For this review, take the finished solid that the model builds, in its own axes (mm). Face numbers are marked on the shaded views. A direction names the side the tool comes from. Give positions to 0.01 mm unless a question says otherwise; leave off trailing zeros. Write each loop counter-clockwise with the first axis right and the second up, starting at its lowest first coordinate (ties: lowest second). Pieces come first, ordered by that corner, then holes. Notation, with made-up numbers: M 61.25,69.25 L 94.25,69.25 A30 ccw 94.25,101.25 Z; hole C 25,-11 d10. An arc over 180 degrees is marked long. Write item = value, one per line.
```python
from build123d import *

# Parameters (mm, degrees)
CHAMFER1_SIZE = 0.5


with BuildPart() as part:
    # Sketch1 → Revolve1 (revolve)
    with BuildSketch(Plane.XY, mode=Mode.PRIVATE) as revolve1_sk:
        Polygon((-99.067365632, -10.161784701), (-100.317365632, -10.161784701), (-100.317365632, -13.161784701), (-92.817365632, -13.161784701), (-92.817365632, 8.038215299), (-97.067365632, 8.038215299), (-97.067365632, 0.538215299), (-99.067365632, 0.538215299), align=None)
    revolve(revolve1_sk.sketch.rotate(Axis((-92.817365632, 8.102615299, 0), (0, -1, 0)), 270), axis=Axis((-92.817365632, 8.102615299, 0), (0, -1, 0)))

    # Chamfer1
    chamfer1_edges = [part.edges().sort_by_distance(p)[0] for p in [
        (-92.817365632, 0.538215299, -6.25),
        (-92.817365632, 8.038215299, -4.25),
    ]]
    chamfer(chamfer1_edges, length=CHAMFER1_SIZE)


solid = part.part
```
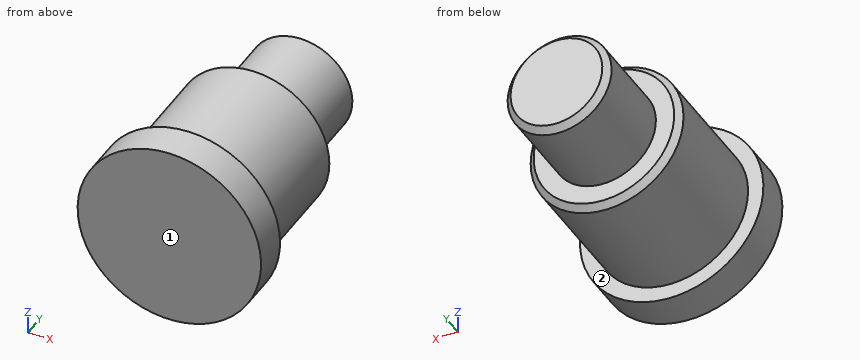
1. We need section A-A, the plane z = 0. Write out the cut boundary in (x, y).
Responses:
outline = M -100.32,-13.16 L -85.32,-13.16 L -85.32,-10.16 L -86.57,-10.16 L -86.57,0.04 L -87.07,0.54 L -88.57,0.54 L -88.57,7.54 L -89.07,8.04 L -96.57,8.04 L -97.07,7.54 L -97.07,0.54 L -98.57,0.54 L -99.07,0.04 L -99.07,-10.16 L -100.32,-10.16 Z
2. For line 1 along Z through (x, y) = (-92.75, -4.5); line 2 along Y through (x, z) = (-88, 0.25); line 3 along Y through (x, z) = (-99.5, 3), list the stretches that pass through material, from the lowest coordinate up. Write a range as from..to.
Responses:
line_1 = -6.25..6.25
line_2 = -13.16..0.54
line_3 = -13.16..-10.16
3. Insertion check: P1, Ø1, axis at x = -90.5, z = 5, coming from the +Y side; P2, Ø2, axis at y = -1.5, z = 3, coming from the +X side; P3, Ø1.5, axis at x = -98, y = -2, coming from the +Z side. Each pin has a flat end and moves straight along its axis. Give the tip position at first contact, or say it passes through.
Responses:
P1 = 0.54
P2 = -86.9
P3 = 4.41
4. Machinability: for the marked faces 1 and 2, which of the approach directions +Z, -Z, +X, -X, +Y, -Y give a long, thin tool a straight path to every point of the face, cutting with its end or side? Answer none if there is none.
Responses:
face_1 = +Z, -Z, +X, -X, -Y
face_2 = +Y
5. We need section B-B, the plane y = -9.25. Write out the cut boundary in (x, z).
Responses:
outline = C -92.82,0 d12.5
6. We need section C-C, the plane y = -11.5. Write out the cut boundary in (x, z).
Responses:
outline = C -92.82,0 d15
